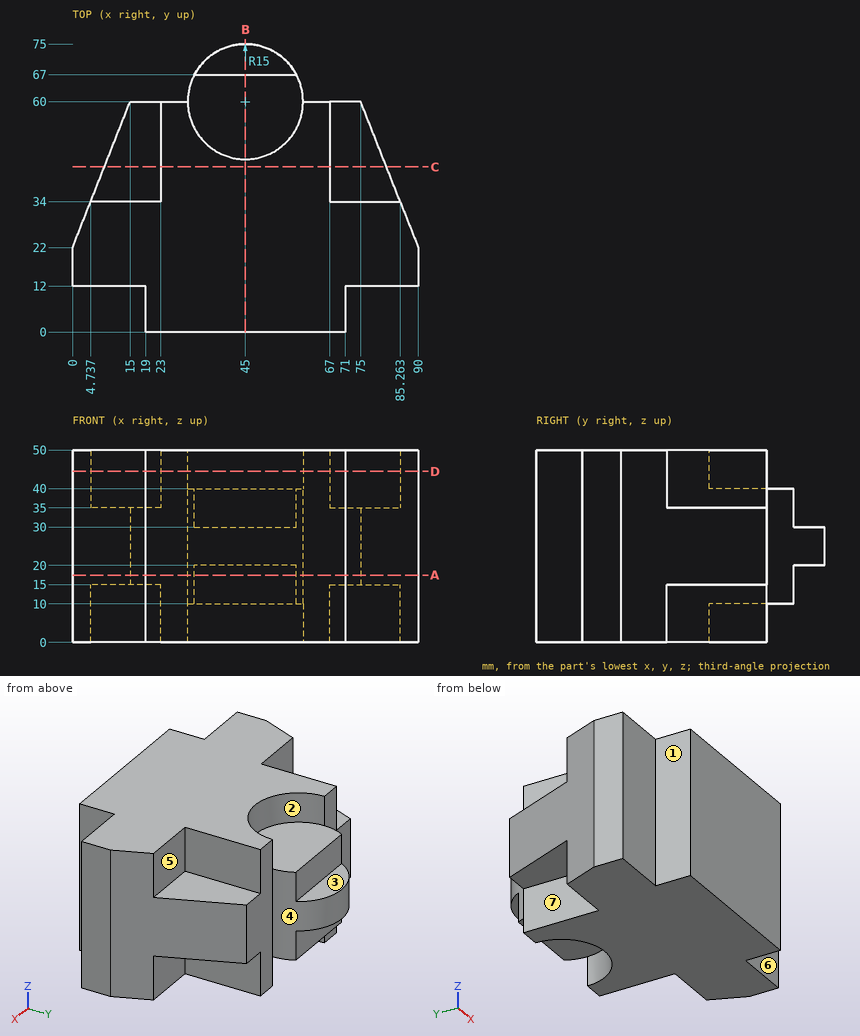
The drawing under review shows one solid part. Ordinate dimensions are in mm from its lowest x, y, z. A direction names the side the tool comes from. Round coordinates to 2 decimals unless told otherwise and drop trailing zeros. Loops run counter-clockwise (first coordinate to the right, second up) from the corner with the lowest first, then second, coordinate; pieces in that order, holes last. Notation, with made-up numbers: (45, 60.25) - (73, 60.25) arc R7 cw to (73, 73.25) - close; hole circle Ø1 at (-25, 18.5). An arc over 180 degrees is marked (long way). One line per question, with ' | ' between items.
Q1. The part is to be moulded in two halves that separate along X. For the marked faces 1, 2, 3 and 4, say which applies: released by +X, released by -X, zero draft, split by the parting line, or undercut.
Taken from the geometry:
face 1: released by -X | face 2: undercut | face 3: zero draft | face 4: split by the parting line
Q2. For line 1 along X through (y, z) = (4, 29); line 2 along Y through (x, z) = (35.5, 34); line 3 along Z through (x, y) = (82, 35.5), list the stretches that pass through material, from the lowest coordinate up. Write a range as [from, to].
Taken from the geometry:
line 1: x = [19, 71] | line 2: y = [0, 67] | line 3: z = [15, 35]
Q3. For pin 1 (9 mm diameter, centred on x = 77.5, y = 49.5, fed in from +Z); pin 2 (6 mm diameter, centred on y = 62, z = 16.5, fed in from +X) (1 decimal); pin 3 (3 mm diameter, centred on x = 47, z = 13.5, fed in from +Y), all flat-tipped, find the tip position at first contact; note any pin that passes through.
Taken from the geometry:
pin 1: stops at z = 35 | pin 2: stops at x = 75.4 | pin 3: stops at y = 67
Q4. Take a section at B-B (x = 45). Give the boundary of the cut face in (y, z).
Taken from the geometry:
outline: (0, 0) - (45, 0) - (45, 10) - (67, 10) - (67, 20) - (75, 20) - (75, 30) - (67, 30) - (67, 40) - (45, 40) - (45, 50) - (0, 50) - close
Q5. Take a section at C-C (y = 43). Give the boundary of the cut face in (x, z).
Taken from the geometry:
outline: (8.29, 15) - (23, 15) - (23, 0) - (67, 0) - (67, 15) - (81.71, 15) - (81.71, 35) - (67, 35) - (67, 50) - (23, 50) - (23, 35) - (8.29, 35) - close
Q6. Take a section at D-D (z = 44.5). Give the boundary of the cut face in (x, y).
Taken from the geometry:
outline: (0, 12) - (19, 12) - (19, 0) - (71, 0) - (71, 12) - (90, 12) - (90, 22) - (85.26, 34) - (67, 34) - (67, 60) - (60, 60) arc R15 cw to (30, 60) - (23, 60) - (23, 34) - (4.74, 34) - (0, 22) - close
Q7. Tool access review of the marked faces 5, 6 and 7: name each direction out of +Z, -Z, +X, -X, +Y, -Y from which nothing blocks a thin tool from reaching the whole face with its end or side.
Taken from the geometry:
face 5: +Z, +X, +Y | face 6: +Z, -Z, +X, -Y | face 7: -Z, -X, +Y
Q8. Take a section at A-A (z = 17.5). Give the boundary of the cut face in (x, y).
Taken from the geometry:
outline: (0, 12) - (19, 12) - (19, 0) - (71, 0) - (71, 12) - (90, 12) - (90, 22) - (75, 60) - (60, 60) arc R15 ccw to (58.27, 67) - (31.73, 67) arc R15 ccw to (30, 60) - (15, 60) - (0, 22) - close
